Geometry: final body of the model. Coordinates: model frame, mm. A direction names the side the tool comes from. Give positions to 0.01 mm unless a question says otherwise; leave off trailing zeros. Write each loop counter-clockwise with the first axis right and the second up, starting at its lowest first coordinate (ties: lowest second). Pieces come first, ordered by that corner, then holes. Notation, with made-up numbers: M 85.25,88 L 100.25,88 A34 ccw 100.25,125 Z; hole C 6,-32 d3. An arc over 180 degrees is marked long. Answer as a JSON object with one key per item and string values.
from build123d import *

# Parameters (mm, degrees)
EXTRUDE_THIN1_DEPTH  = 100
SKETCH2_R            = 5
CUT_EXTRUDE1_DEPTH   = 10
LPATTERN1_COUNT      = 2
LPATTERN1_PITCH      = 400
LPATTERN1_COUNT_DIR2 = 2
LPATTERN1_PITCH_DIR2 = 70


with BuildPart() as part:
    # Sketch1 → Extrude-Thin1 (new body)
    with BuildSketch(Plane.XY):
        with BuildLine():
            Line((0, 0), (0, 120))
            ThreePointArc((0, 120), (8.786796564, 141.213203436), (30, 150))
            Line((30, 150), (648, 150))
            Line((648, 150), (648, 145))
            Line((648, 145), (30, 145))
            ThreePointArc((30, 145), (12.32233047, 137.67766953), (5, 120))
            Line((5, 120), (5, 0))
            Line((5, 0), (0, 0))
        make_face()
    extrude(amount=EXTRUDE_THIN1_DEPTH)

    # Sketch2 → Cut-Extrude1 (cut)
    with BuildSketch(Plane.XZ.offset(-145)):
        with Locations(Location((55, 85, 0), (0, 0, 270))):
            Circle(SKETCH2_R)
    cut_extrude1 = extrude(amount=-CUT_EXTRUDE1_DEPTH, mode=Mode.SUBTRACT)

    # LPattern1: Cut-Extrude1 2 × 2
    with Locations(*[(i * LPATTERN1_PITCH, 0, -j * LPATTERN1_PITCH_DIR2) for i in range(LPATTERN1_COUNT) for j in range(LPATTERN1_COUNT_DIR2) if (i, j) != (0, 0)]):
        add(cut_extrude1, mode=Mode.SUBTRACT)


solid = part.part
1) Cut plane A-A on z = 31.5. Return loops of the section in (x, y).
Geometry check:
{"outline": "M 0,0 L 5,0 L 5,120 A25 cw 30,145 L 648,145 L 648,150 L 30,150 A30 ccw 0,120 Z"}
2) Cut plane C-C on y = 58.5. Return loops of the section in (x, z), and give its area (3 significant figures).
Geometry check:
{"outline": "M 0,0 L 5,0 L 5,100 L 0,100 Z", "area": "500 mm2"}
3) Contact query for flat-ended pins moving along their axis: P1, Ø8, axis at x = 55, z = 85, coming from the +Y side; P2, Ø3, axis at y = 58, z = 67, coming from the +X side; P3, Ø16, axis at x = 455, z = 15, coming from the -Y side. Output: stop coordinate, or through.
Geometry check:
{"P1": "passes through", "P2": "stops at x = 5", "P3": "stops at y = 145"}
4) Line query: line 1 (Z direction, x = 455, y = 148.65); line 2 (X direction, y = 146.4, z = 15); line 3 (Y direction, x = 579, z = 70.5). Output: solid intervals per line, ascending. Write a range as from..to.
Geometry check:
{"line 1": "z = 0..10, 20..80, 90..100", "line 2": "x = 15.75..50, 60..450, 460..648", "line 3": "y = 145..150"}
5) Set-up query: faces 1 (the flat face through (343, 145, 49)), 2 (the cylindrical face through (8.555, 140.979, 49.3)). Return all of +Z, -Z, +X, -X, +Y, -Y with unobstructed straight access to the full face (end or side cutting, diameter ignored); none if empty.
Geometry check:
{"face 1": "+Z, -Z, +X, -Y", "face 2": "+Z, -Z, -X, +Y"}
6) Cut plane B-B on x = 274. Return loops of the section in (y, z), and give its area (3 significant figures).
Geometry check:
{"outline": "M 145,0 L 150,0 L 150,100 L 145,100 Z", "area": "500 mm2"}
